from build123d import *

# Parameters (mm, degrees)
SKETCH1_W                                           = 100
SKETCH1_H                                           = 55
BOSS_EXTRUDE1_DEPTH                                 = 12
SKETCH2_W                                           = 65
SKETCH2_H                                           = 12
BOSS_EXTRUDE2_DEPTH                                 = 12
CBORE_FOR_M4_HEX_SOCKET_HEAD_CAP_SCREW1_D           = 4.5
CBORE_FOR_M4_HEX_SOCKET_HEAD_CAP_SCREW1_CBORE_D     = 8
CBORE_FOR_M4_HEX_SOCKET_HEAD_CAP_SCREW1_CBORE_DEPTH = 4.4
CHAMFER1_SIZE                                       = 40
CHAMFER1_SIZE2                                      = 20
CHAMFER2_SIZE                                       = 20
CHAMFER2_SIZE2                                      = 40


with BuildPart() as part:
    # Sketch1 → Boss-Extrude1 (new body)
    with BuildSketch(Plane.XY):
        Rectangle(SKETCH1_W, SKETCH1_H)
    extrude(amount=BOSS_EXTRUDE1_DEPTH)

    # Sketch2 → Boss-Extrude2 (add)
    with BuildSketch(Plane.XZ.offset(27.5)):
        with Locations((0, 6)):
            Rectangle(SKETCH2_W, SKETCH2_H)
    extrude(amount=BOSS_EXTRUDE2_DEPTH)

    # CBORE for M4 Hex Socket Head Cap Screw1 (through all)
    with Locations(Plane(origin=(0, 0, 0), x_dir=(-1, 0, 0), z_dir=(0, 0, -1))):
        with Locations((15, -33.5), (-15, -33.5)):
            CounterBoreHole(CBORE_FOR_M4_HEX_SOCKET_HEAD_CAP_SCREW1_D / 2, CBORE_FOR_M4_HEX_SOCKET_HEAD_CAP_SCREW1_CBORE_D / 2, CBORE_FOR_M4_HEX_SOCKET_HEAD_CAP_SCREW1_CBORE_DEPTH)

    # Chamfer1
    chamfer1_edges = [part.edges().sort_by_distance(p)[0] for p in [
        (50, 27.5, 6),
    ]]
    chamfer1_side = [part.faces().sort_by_distance(p)[0] for p in [
        (50, 0, 6),
    ]]
    chamfer(chamfer1_edges, length=CHAMFER1_SIZE, length2=CHAMFER1_SIZE2, reference=chamfer1_side[0])

    # Chamfer2
    chamfer2_edges = [part.edges().sort_by_distance(p)[0] for p in [
        (-50, 27.5, 6),
    ]]
    chamfer2_side = [part.faces().sort_by_distance(p)[0] for p in [
        (-10, 27.5, 6),
    ]]
    chamfer(chamfer2_edges, length=CHAMFER2_SIZE, length2=CHAMFER2_SIZE2, reference=chamfer2_side[0])


solid = part.part
For this review, take the finished solid that the model builds, in its own axes (mm). A direction names the side the tool comes from. Coordinates: 2 decimals unless noted, no trailing zeros. Write each loop counter-clockwise with the first axis right and the second up, starting at its lowest first coordinate (ties: lowest second). Pieces come first, ordered by that corner, then holes. Notation, with made-up numbers: (51.5, 51) -> (55.5, 51) arc R20 ccw to (55.5, 74) -> close; hole circle Ø10 at (19, 23.5). An arc over 180 degrees is marked (long way). Write each question's results on one line, items separated by ' | '. Start each with the question number.
1) Consider section B-B (x = 15). Write out the cut boundary in (y, z).
2) Insertion check: pin 1 (6 mm diameter, centred on y = 18, z = 8, fed in from +X); pin 2 (3.5 mm diameter, centred on x = 40.5, z = 3, fed in from -Y); pin 3 (1.5 mm diameter, centred on x = -36.5, z = 6.5, fed in from +Y); pin 4 (2.5 mm diameter, centred on x = -15, y = -33.5, fed in from +Z). Each pin has a flat end and moves straight along its axis. Give the tip position at first contact, or say it passes through.
3) Consider section A-A (z = 8.75). Write out the cut boundary in (x, y).
4) Consider section C-C (y = -33.5). Write out the cut boundary in (x, z).
5) The part is to be moulded in two halves that separate along X. For faces 6 (the face through (50, -20, 6)), 7 (the face through (16.21, -31.603, 8.253)), 8 (the face through (-41, -27.5, 6)), say which applies: +X half, -X half, draft (parallel to the pull), parting line (faces both ways), or undercut.
6) For faces 1 (the face through (0, 27.5, 6)), 2 (the face through (13, -35, 4.4)), 3 (the face through (-32.5, -33, 6)), 4 (the face through (32.5, -33, 6)), 5 (the face through (-50, -20, 6)), list the 3-axis set-ups (+Z, -Z, +X, -X, +Y, -Y) from which the entire face can be reached by the end or side of a thin tool; tool diameter is ignored.
7) Wall thickness on L1, parallel to Y at x = 15, z = 2.5; L2, parallel to X at y = -35.5, z = 5; L3, parallel to X at y = -32, z = 1: over which ranges is each line inside the solid? List them lowest first. Write a range as [from, to].
8) Consider section D-D (z = 3.25). Write out the cut boundary in (x, y).
Geometry says:
1) outline: (-39.5, 0) -> (-37.5, 0) -> (-37.5, 4.4) -> (-35.75, 4.4) -> (-35.75, 12) -> (-39.5, 12) -> close; (-31.25, 4.4) -> (-29.5, 4.4) -> (-29.5, 0) -> (27.5, 0) -> (27.5, 12) -> (-31.25, 12) -> close
2) pin 1: x = 36.25 | pin 2: y = -27.5 | pin 3: y = 16 | pin 4: through
3) outline: (-50, -27.5) -> (-32.5, -27.5) -> (-32.5, -39.5) -> (32.5, -39.5) -> (32.5, -27.5) -> (50, -27.5) -> (50, -12.5) -> (30, 27.5) -> (-30, 27.5) -> (-50, -12.5) -> close; hole circle Ø4.5 at (-15, -33.5); hole circle Ø4.5 at (15, -33.5)
4) outline: (-32.5, 0) -> (-19, 0) -> (-19, 4.4) -> (-17.25, 4.4) -> (-17.25, 12) -> (-32.5, 12) -> close; (-12.75, 4.4) -> (-11, 4.4) -> (-11, 0) -> (11, 0) -> (11, 4.4) -> (12.75, 4.4) -> (12.75, 12) -> (-12.75, 12) -> close; (17.25, 4.4) -> (19, 4.4) -> (19, 0) -> (32.5, 0) -> (32.5, 12) -> (17.25, 12) -> close
5) face 6: +X half | face 7: undercut | face 8: draft
6) face 1: +Z, -Z, +X, -X, +Y | face 2: -Z | face 3: +Z, -Z, -X, -Y | face 4: +Z, -Z, +X, -Y | face 5: +Z, -Z, -X, +Y, -Y
7) L1: [-39.5, -37.5], [-29.5, 27.5] | L2: [-32.5, -16.03], [-13.97, 13.97], [16.03, 32.5] | L3: [-32.5, -18.71], [-11.29, 11.29], [18.71, 32.5]
8) outline: (-50, -27.5) -> (-32.5, -27.5) -> (-32.5, -39.5) -> (32.5, -39.5) -> (32.5, -27.5) -> (50, -27.5) -> (50, -12.5) -> (30, 27.5) -> (-30, 27.5) -> (-50, -12.5) -> close; hole circle Ø8 at (-15, -33.5); hole circle Ø8 at (15, -33.5)
